Here's how the part is built. I have some questions about the finished solid (model axes, mm). A direction names the side the tool comes from. Coordinates: 2 decimals unless noted, no trailing zeros. Write each loop counter-clockwise with the first axis right and the second up, starting at its lowest first coordinate (ties: lowest second). Pieces come first, ordered by that corner, then holes.
(1) Imagine slicing it at C-C, the plane y = 2. List the corners of the cut face in (x, z) for me.
(2) Imagine slicing it at D-D, the plane x = -7.25. List the corners of the cut face in (y, z) for me.
(3) Thinking about a two-plate mould opening in Y: for faces 1 (the cylindrical face through (9.7, -23.04, 6.18)), 2 (the cylindrical face through (-3.755, -27.479, -11.923)), 3 (the flat face through (0, 29, 0)), 4 (the flat face through (0, -29, 0)), which applies, released by +Y, released by -Y, zero draft, split by the parting line, or undercut?
(4) For pin 1 Ø1 at (y, z) = (-0.5, 9) entering from +X; pin 2 Ø4 at (y, z) = (20, 5.5) entering from -X; pin 3 Ø6 at (y, z) = (22.5, -7) entering from -X, each with a flat end and sliding along its axis, tell me the tip position at first contact or that it passes through.
(5) Which directions (+Z, -Z, +X, -X, +Y, -Y) give clear straight access to the entire face, cutting with the end or side of a thin tool? Please do faces 5 (the cylindrical face through (7.606, 0.28, 9.92)), 6 (the flat face through (11, -26, -4)), 7 (the flat face through (0, -12.5, -8)).
(6) Please list where these lines run through material, in increasing order: probe 1 along Y at (x, z) = (-0.25, -7.5); probe 2 along Y at (x, z) = (0, 2); probe 3 along X at (y, z) = (0, -0.5).
(7) Imagine slicing it at B-B, the plane z = 0. List the corners of the cut face in (x, y) for me.
(8) Imagine slicing it at A-A, the plane x = 0. List the corners of the cut face in (y, z) for me, plus the area to 3 significant figures.
```python
from build123d import *

# Parameters (mm, degrees)
SKETCH1_R           = 12.5
BOSS_EXTRUDE1_DEPTH = 29
CUT_EXTRUDE1_START  = -3
SKETCH2_R           = 12.5
SKETCH2_R_2         = 11.5
CUT_EXTRUDE1_DEPTH  = 6
SKETCH3_W           = 7
SKETCH3_H           = 25
CUT_EXTRUDE2_DEPTH  = 33
SKETCH4_R           = 6.5
CUT_EXTRUDE3_DEPTH  = 37.349002737


with BuildPart() as part:
    # Sketch1 → Boss-Extrude1 (new, symmetric)
    with BuildSketch(Plane(origin=(0, 0, 0), x_dir=(1, 0, 0), z_dir=(0, 1, 0))):
        with Locations(Location((0, 0, 0), (0, 0, 90))):
            Circle(SKETCH1_R)
    extrude(amount=BOSS_EXTRUDE1_DEPTH, both=True)

    # Sketch2 → Cut-Extrude1 (cut)
    with BuildSketch(Plane(origin=(0, 29, 0), x_dir=(1, 0, 0), z_dir=(0, 1, 0)).offset(CUT_EXTRUDE1_START)):
        with Locations(Location((0, 0, 0), (0, 0, 90))):
            Circle(SKETCH2_R)
        with Locations(Location((0, 0, 0), (0, 0, 270))):
            Circle(SKETCH2_R_2, mode=Mode.SUBTRACT)
    cut_extrude1 = extrude(amount=-CUT_EXTRUDE1_DEPTH, mode=Mode.SUBTRACT)

    # Mirror1: Cut-Extrude1 across plane
    add(cut_extrude1.mirror(Plane.ZX), mode=Mode.SUBTRACT)

    # Sketch3 → Cut-Extrude2 (cut, symmetric)
    with BuildSketch(Plane(origin=(0, 0, 0), x_dir=(0, 0, -1), z_dir=(1, 0, 0))):
        with Locations((9, 0)):
            Rectangle(SKETCH3_W, SKETCH3_H)
    extrude(amount=CUT_EXTRUDE2_DEPTH, both=True, mode=Mode.SUBTRACT)

    # Sketch4 → Cut-Extrude3 (cut, through all)
    with BuildSketch(Plane(origin=(0, 0, -5.5), x_dir=(-1, 0, 0), z_dir=(0, 0, -1))):
        with Locations(Location((0, 0, 0), (0, 0, 90))):
            Circle(SKETCH4_R)
    extrude(amount=-CUT_EXTRUDE3_DEPTH, mode=Mode.SUBTRACT)


solid = part.part
```
Recorded:
1. outline: (-11.22, -5.5) - (-6.18, -5.5) - (-6.18, 10.86) arc R12.5 ccw to start; (6.18, -5.5) - (11.22, -5.5) arc R12.5 ccw to (6.18, 10.86) - close
2. outline: (-29, -10.18) - (-26, -10.18) - (-26, -8.93) - (-20, -8.93) - (-20, -10.18) - (-12.5, -10.18) - (-12.5, -5.5) - (12.5, -5.5) - (12.5, -10.18) - (20, -10.18) - (20, -8.93) - (26, -8.93) - (26, -10.18) - (29, -10.18) - (29, 10.18) - (26, 10.18) - (26, 8.93) - (20, 8.93) - (20, 10.18) - (-20, 10.18) - (-20, 8.93) - (-26, 8.93) - (-26, 10.18) - (-29, 10.18) - close
3. face 1: undercut
3. face 2: zero draft
3. face 3: released by +Y
3. face 4: released by -Y
4. pin 1: stops at x = 9.17
4. pin 2: stops at x = -12
4. pin 3: stops at x = -11.3
5. face 5: +Y, -Y
5. face 6: none
5. face 7: -Z, +X, -X
6. probe 1: y = -29 to -12.5, 12.5 to 29
6. probe 2: y = -29 to -6.5, 6.5 to 29
6. probe 3: x = -12.49 to -6.5, 6.5 to 12.49
7. outline: (-12.5, -29) - (12.5, -29) - (12.5, -26) - (11.5, -26) - (11.5, -20) - (12.5, -20) - (12.5, 20) - (11.5, 20) - (11.5, 26) - (12.5, 26) - (12.5, 29) - (-12.5, 29) - (-12.5, 26) - (-11.5, 26) - (-11.5, 20) - (-12.5, 20) - (-12.5, -20) - (-11.5, -20) - (-11.5, -26) - (-12.5, -26) - close; hole circle Ø13 at (0, 0)
8. outline: (-29, -12.5) - (-26, -12.5) - (-26, -11.5) - (-20, -11.5) - (-20, -12.5) - (-12.5, -12.5) - (-12.5, -5.5) - (-6.5, -5.5) - (-6.5, 12.5) - (-20, 12.5) - (-20, 11.5) - (-26, 11.5) - (-26, 12.5) - (-29, 12.5) - close; (6.5, -5.5) - (12.5, -5.5) - (12.5, -12.5) - (20, -12.5) - (20, -11.5) - (26, -11.5) - (26, -12.5) - (29, -12.5) - (29, 12.5) - (26, 12.5) - (26, 11.5) - (20, 11.5) - (20, 12.5) - (6.5, 12.5) - close
8. area: 1,020 mm2
